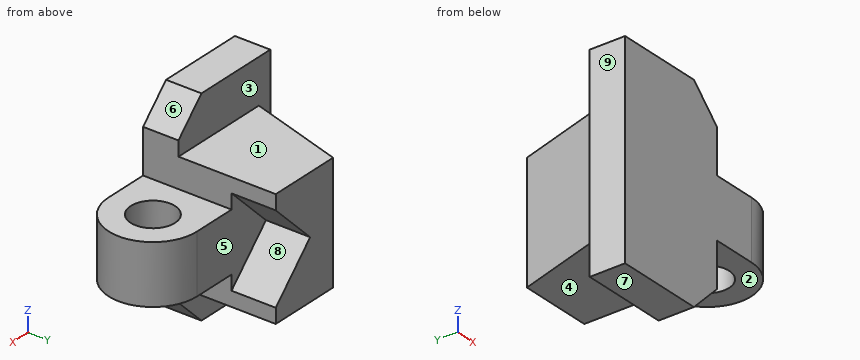
```python
from build123d import *

# Parameters (mm, degrees)
BRACKET_PROFILE_SKETCH_R       = 7.5
LUG_EYE_BOSS_20MM_DEPTH        = 10
SKETCH5_3_W                    = 40
SKETCH5_3_H                    = 12
BASE_BLOCK_70MM_DEPTH          = 35
UPRIGHT_BLOCK_40MM_DEPTH       = 20
UPRIGHT_EDGE_CHAMFER_10MM_SIZE = 10
FORK_SLOT_CUT_30X15_DEPTH      = 15


with BuildPart() as part:
    # Bracket Profile Sketch → Lug Eye Boss 20mm (new, symmetric)
    with BuildSketch(Plane.XY):
        with BuildLine():
            Line((-15, -3), (-15, -15))
            Line((-15, -15), (0, -15))
            ThreePointArc((0, -15), (15, 0), (0, 15))
            Line((0, 15), (-15, 15))
            Line((-15, 15), (-15, -3))
        make_face()
        Circle(BRACKET_PROFILE_SKETCH_R, mode=Mode.SUBTRACT)
    extrude(amount=LUG_EYE_BOSS_20MM_DEPTH, both=True)

    # Sketch5_3 → Base Block 70mm (add, symmetric)
    with BuildSketch(Plane.XY):
        with Locations((-35, -9)):
            Rectangle(SKETCH5_3_W, SKETCH5_3_H)
    extrude(amount=BASE_BLOCK_70MM_DEPTH, both=True)

    # Sketch5_4 → Upright Block 40mm (add, symmetric)
    with BuildSketch(Plane.XY):
        Polygon((-50, -3), (-15, -3), (-15, 15), (-15, 30), (-40, 30), align=None)
    extrude(amount=UPRIGHT_BLOCK_40MM_DEPTH, both=True)

    # Upright Edge Chamfer 10mm
    upright_edge_chamfer_10mm_edges = [part.edges().sort_by_distance(p)[0] for p in [
        (-15, -9, -35),
        (-15, -9, 35),
    ]]
    chamfer(upright_edge_chamfer_10mm_edges, length=UPRIGHT_EDGE_CHAMFER_10MM_SIZE)

    # Fork Slot Sketch → Fork Slot Cut 30x15 (cut)
    with BuildSketch(Plane(origin=(0, 30, 0), x_dir=(1, 0, 0), z_dir=(0, 1, 0))):
        Polygon((-15, -15), (-30, 0), (-15, 15), align=None)
    extrude(amount=-FORK_SLOT_CUT_30X15_DEPTH, mode=Mode.SUBTRACT)


solid = part.part
```
Can you work these out from the model? Positions are in its coordinate system, mm. Face numbers are marked on the shaded views. A direction names the side the tool comes from. Coordinates: 2 decimals unless noted, no trailing zeros. Loops run counter-clockwise (first coordinate to the right, second up) from the corner with the lowest first, then second, coordinate; pieces in that order, holes last.
1) Imagine slicing it at A-A on z = 3. List the corners of the cut face in (x, y) for me.
2) Which directions (+Z, -Z, +X, -X, +Y, -Y) give clear straight access to the entire face, cutting with the end or side of a thin tool? Please do the marked faces 1, 2, 3, 4 and 5.
3) I need wall thicknesses on probe 1 along X at (y, z) = (-11, 16); probe 2 along Z at (x, y) = (2, -10); probe 3 along Y at (x, z) = (-47.5, -28). Which ranges of each line are inside material? Lowest first, please.
4) For pin 1 (4.5 mm diameter, centred on y = 10.5, z = 14, fed in from +X); pin 2 (4 mm diameter, centred on y = 8, z = -8, fed in from -X); pin 3 (13.5 mm diameter, centred on x = 0, y = 0, fed in from -Z); pin 4 (9 mm diameter, centred on x = -2.5, y = 3, fed in from +Z), each with a flat end and sliding along its axis, tell me the tip position at first contact or that it passes through.
5) Imagine slicing it at D-D on x = -5. List the corners of the cut face in (y, z) for me, plus the area to 3 significant figures.
6) Imagine slicing it at B-B on x = -19.5. List the corners of the cut face in (y, z) for me.
7) Imagine slicing it at C-C on y = 0. List the corners of the cut face in (x, z) for me.
8) Thinking about a two-plate mould opening in Z: for the marked faces 6, 7, 8 and 9, which applies, pulls with the +Z half, pulls with the -Z half, needs draft (parallel to the pull), parting line crosses it, or undercut?
Completed:
1. outline: (-55, -15) - (0, -15) arc R15 ccw to (0, 15) - (-27, 15) - (-27, 30) - (-40, 30) - (-50, -3) - (-55, -3) - close; hole circle Ø15 at (0, 0)
2. face 1: +Z, +X, -X, +Y
2. face 2: -Z, +X, +Y, -Y
2. face 3: -X, +Y
2. face 4: -Z, +X, -X, +Y
2. face 5: +X, +Y
3. probe 1: x = -55 to -15
3. probe 2: z = -10 to 10
3. probe 3: y = -15 to -3
4. pin 1: stops at x = -15
4. pin 2: stops at x = -47.27
4. pin 3: passes through
4. pin 4: stops at z = 10
5. outline: (-15, -10) - (-5.59, -10) - (-5.59, 10) - (-15, 10) - close; (5.59, -10) - (15, -10) - (15, 10) - (5.59, 10) - close
5. area: 376 mm2
6. outline: (-15, -29.5) - (-3, -29.5) - (-3, -20) - (30, -20) - (30, -10.5) - (15, -10.5) - (15, 10.5) - (30, 10.5) - (30, 20) - (-3, 20) - (-3, 29.5) - (-15, 29.5) - close
7. outline: (-49.09, -20) - (-15, -20) - (-15, -10) - (-7.5, -10) - (-7.5, 10) - (-15, 10) - (-15, 20) - (-49.09, 20) - close; (7.5, -10) - (15, -10) - (15, 10) - (7.5, 10) - close
8. face 6: pulls with the +Z half
8. face 7: pulls with the -Z half
8. face 8: undercut
8. face 9: needs draft
